Here's the drawing with two shaded views (mm, measured from the low corner). I have some questions. A direction names the side the tool comes from. Round coordinates to 2 decimals unless told otherwise and drop trailing zeros. Loops run counter-clockwise (first coordinate to the right, second up) from the corner with the lowest first, then second, coordinate; pieces in that order, holes last.
(1) I want a section at B-B on y = 39.5. Write out the boundary of the cut face in (x, z).
(2) Thinking about a two-plate mould opening in Z: for the marked faces 6, 7, 8 and 9, which applies, released by +Z, released by -Z, zero draft, split by the parting line, or undercut?
(3) Will these pins go through, and if not, where does the flat tip stop? pin 1 Ø20 at (x, z) = (26, 73) entering from -Y; pin 2 Ø14.5 at (x, y) = (11, 21) entering from +Z; pin 3 Ø12 at (x, y) = (7, 28.5) entering from -Z; pin 4 Ø6 at (y, z) = (12, 25) entering from -X.
(4) Which directions (+Z, -Z, +X, -X, +Y, -Y) give clear straight access to the entire face, cutting with the end or side of a thin tool? Please do the marked faces 1, 2, 3, 4 and 5.
(5) If I drill on line 1 along X through (y, z) = (64.5, 32.5); line 2 along Y through (x, z) = (48.75, 25); line 3 along Y through (x, z) = (19.5, 14), over which ranges is the centre line in solid material (lowest first)?
(6) I want a section at D-D on x = 19.5. Write out the boundary of the cut face in (y, z).
(7) I want a section at C-C on z = 82.5. Write out the boundary of the cut face in (x, y), plus the area to 3 significant figures.
(8) I want a section at A-A on y = 8.5. Write out the boundary of the cut face in (x, z), plus the area to 3 significant figures.
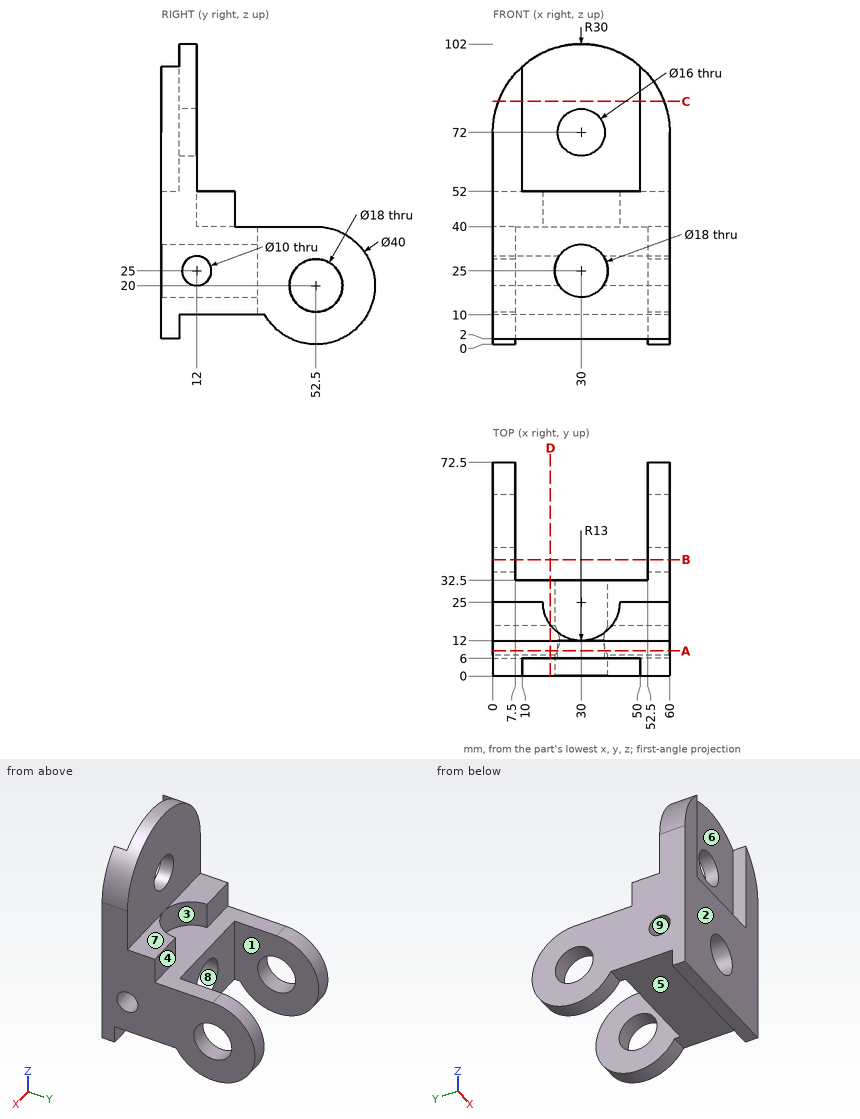
Filled sheet:
1. outline: (0, 4.8) - (7.5, 4.8) - (7.5, 40) - (0, 40) - close; (52.5, 4.8) - (60, 4.8) - (60, 40) - (52.5, 40) - close
2. face 6: zero draft
2. face 7: released by +Z
2. face 8: undercut
2. face 9: undercut
3. pin 1: stops at y = 6
3. pin 2: stops at z = 52
3. pin 3: stops at z = 10
3. pin 4: passes through
4. face 1: +Z, -Z, +Y
4. face 2: +Z, -Z, +X, -X, -Y
4. face 3: +Z, +Y
4. face 4: +Z, +X, -X, +Y
4. face 5: -Z, +X, -X
5. line 1: x = 0 to 7.5, 52.5 to 60
5. line 2: y = 0 to 7, 17 to 32.5
5. line 3: y = 0 to 32.5
6. outline: (0, 2) - (6, 2) - (6, 10) - (32.5, 10) - (32.5, 40) - (17.34, 40) - (17.34, 52) - (12, 52) - (12, 100.1) - (6, 100.1) - (6, 52) - (0, 52) - close; hole circle Ø10 at (12, 25)
7. outline: (1.9, 0) - (10, 0) - (10, 6) - (50, 6) - (50, 0) - (58.1, 0) - (58.1, 12) - (1.9, 12) - close
7. area: 434 mm2
8. outline: (0, 10) - (60, 10) - (60, 21.43) - (38.26, 21.43) arc R9 cw to (21.74, 21.43) - (0, 21.43) - close; (0, 28.57) - (21.74, 28.57) arc R9 cw to (38.26, 28.57) - (60, 28.57) - (60, 72) arc R30 ccw to (0, 72) - close; hole circle Ø16 at (30, 72)
8. area: 4,370 mm2
